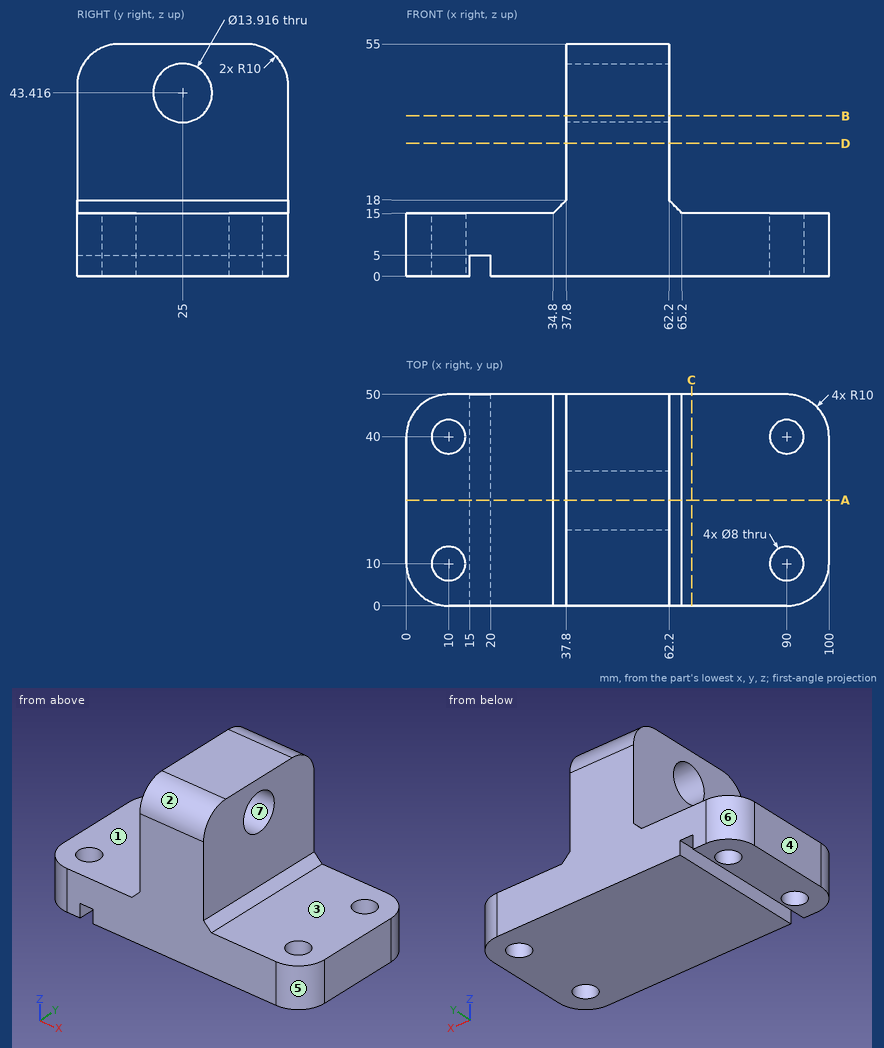
Could you check a few things on this drawing? It's one solid part, dimensions in mm from its lowest x, y, z. A direction names the side the tool comes from. Give positions to 0.01 mm unless a question says otherwise; leave off trailing zeros. Order: outer loops, then holes, each group sorted by start corner. A loop starts at its lowest first (then second) coordinate and runs counter-clockwise, first axis right, second up. Notation, with made-up numbers: M 39.25,39 L 44.25,39 A25 cw 44.25,52 Z; hole C 84,9 d2. An arc over 180 degrees is marked long. Use one line per item in the form item = value. Start each with the question number.
Item 1: If I drill on line 1 along Z through (x, y) = (79.5, 18.5); line 2 along X through (y, z) = (37.5, 34); line 3 along Y through (x, z) = (89.5, 4.5), over which ranges is the centre line in solid material (lowest first)?
Item 2: If we section it at A-A (y = 25): Write out the boundary of the cut face in (x, z).
Item 3: If we section it at C-C (x = 67.5): Write out the boundary of the cut face in (y, z).
Item 4: If we section it at D-D (z = 31.5): Write out the boundary of the cut face in (x, y), then the cut area to 3 significant figures.
Item 5: If we section it at B-B (z = 38): Write out the boundary of the cut face in (x, y), then the cut area to 3 significant figures.
Item 6: Will these pins go through, and if not, where does the flat tip stop? pin 1 Ø4 at (x, y) = (17.5, 29) entering from -Z; pin 2 Ø12 at (y, z) = (5.5, 35.5) entering from +X; pin 3 Ø5 at (x, y) = (11.5, 29.5) entering from -Z; pin 4 Ø10.5 at (x, y) = (10, 40) entering from +Z.
Item 7: For the marked faces 1, 2 and 3, which set-ups out of +Z, -Z, +X, -X, +Y, -Y let a thin tool reach every point of the face, with its end or its side?
Item 8: We'd pull the mould along Y, two halves only. Please class the marked faces 4, 5, 6 and 7: +Y half, -Y half, draft (parallel to the pull), parting line (faces both ways), or undercut.
Outcome:
q1.line_1 = 0 to 15
q1.line_2 = 37.8 to 62.2
q1.line_3 = 0 to 6.03, 13.97 to 36.03, 43.97 to 50
q2.outline = M 0,0 L 15,0 L 15,5 L 20,5 L 20,0 L 100,0 L 100,15 L 65.2,15 L 62.2,18 L 62.2,36.46 L 37.8,36.46 L 37.8,18 L 34.8,15 L 0,15 Z; M 37.8,50.37 L 62.2,50.37 L 62.2,55 L 37.8,55 Z
q3.outline = M 0,0 L 50,0 L 50,15 L 0,15 Z
q4.outline = M 37.8,0 L 62.2,0 L 62.2,50 L 37.8,50 Z
q4.area = 1,220 mm2
q5.outline = M 37.8,0 L 62.2,0 L 62.2,20.63 L 37.8,20.63 Z; M 37.8,29.37 L 62.2,29.37 L 62.2,50 L 37.8,50 Z
q5.area = 1,010 mm2
q6.pin_1 = 5
q6.pin_2 = 62.2
q6.pin_3 = 0
q6.pin_4 = 15
q7.face_1 = +Z, -X, +Y, -Y
q7.face_2 = +Z, +X, -X, -Y
q7.face_3 = +Z, +X, +Y, -Y
q8.face_4 = draft
q8.face_5 = -Y half
q8.face_6 = +Y half
q8.face_7 = undercut
